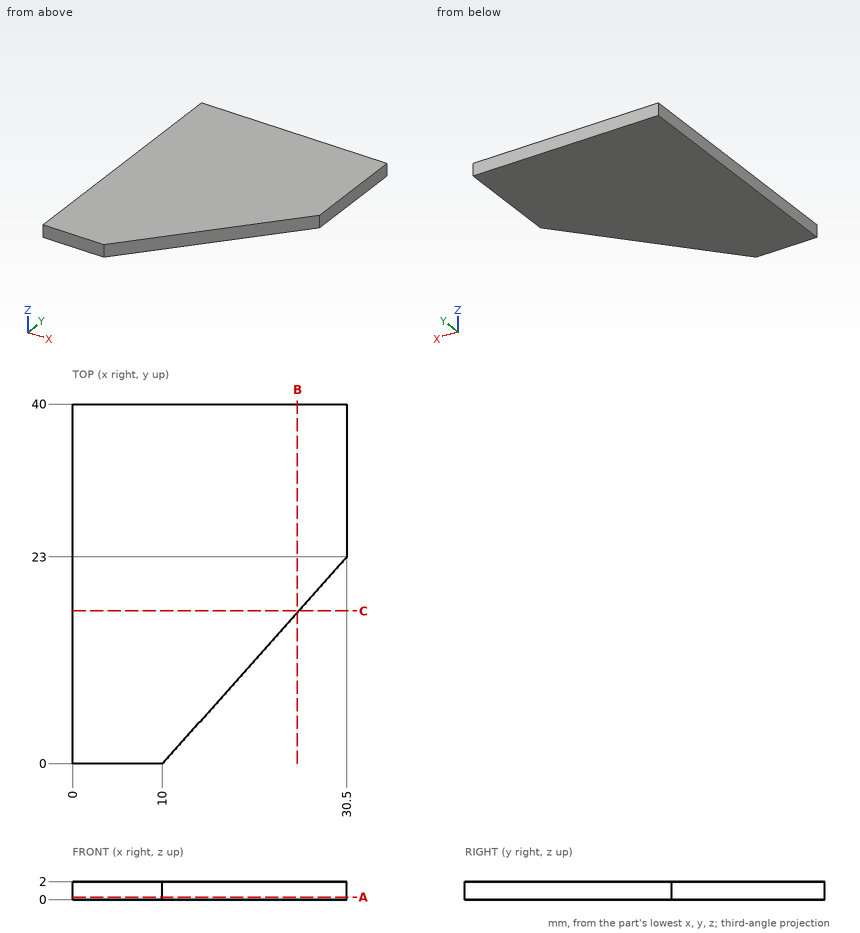
The figure shows three views and two pictorial views of one solid part (mm, origin at its lowest corner). Answer the questions. Coordinates: 2 decimals unless noted, no trailing zeros. Write each loop counter-clockwise with the first axis right and the second up, starting at its lowest first coordinate (ties: lowest second). Pieces come first, ordered by that corner, then holes.
1. Flat-ended cylindrical pins translate along their axes: pin 1 (5 mm diameter, centred on x = 10.5, y = 31, fed in from -Z); pin 2 (1 mm diameter, centred on x = 13.5, z = 0.5, fed in from -Y). Find the tip coordinate at first contact, or state that the pin passes through.
Results list:
pin 1: stops at z = 0
pin 2: stops at y = 3.37
2. Consider line 1 along Y through (x, z) = (24, 1.8); line 2 along Y through (x, z) = (23.5, 0.4); line 3 along X through (y, z) = (6, 1.75). Determine where each line is inside the solid, lowest interval first.
Results list:
line 1: y = 15.71 to 40
line 2: y = 15.15 to 40
line 3: x = 0 to 15.35
3. The part is cut by section A-A, the plane z = 0.3. Write down the section's boundary in (x, y), and give its area (3 significant figures).
Results list:
outline: (0, 0) - (10, 0) - (30.5, 23) - (30.5, 40) - (0, 40) - close
area: 984 mm2
4. The part is cut by section C-C, the plane y = 17. Write down the section's boundary in (x, z), and give its area (3 significant figures).
Results list:
outline: (0, 0) - (25.15, 0) - (25.15, 2) - (0, 2) - close
area: 50.3 mm2
5. The part is cut by section B-B, the plane x = 25. Write down the section's boundary in (y, z), and give its area (3 significant figures).
Results list:
outline: (16.83, 0) - (40, 0) - (40, 2) - (16.83, 2) - close
area: 46.3 mm2
